from build123d import *

# Parameters (mm, degrees)
EXTRUDE_670_DEPTH        = 1730
SKETCH_2_W               = 49
SKETCH_2_H               = 55.5
EXTRUDE_1_DEPTH          = 85
SKETCH_4_W               = 49
SKETCH_4_H               = 55.5
EXTRUDE_3_DEPTH          = 95
SKETCH_9_R               = 23.5
CUT_EXTRUDE_5_DEPTH      = 3
SKETCH_10_R              = 6
EXTRUDE_4_DEPTH          = 28
CHAMFER_1_SIZE           = 1
PATTERN_CIRCULAR_1_COUNT = 4


with BuildPart() as part:
    # 草图1 → Extrude 670 (new body)
    with BuildSketch(Plane.XY):
        Polygon((15, 50), (15, 42), (35, 42), (35, 50), (50, 50), (50, 20), (42, 20), (42, 10), (50, 10), (50, 0), (0, 0), (0, 10), (8, 10), (8, 20), (0, 20), (0, 50), align=None)
    extrude(amount=EXTRUDE_670_DEPTH)

    # 草图2 → 凸台-拉伸1 (add)
    with BuildSketch(Plane.XY.offset(1730)):
        with Locations((25, 27.75)):
            Rectangle(SKETCH_2_W, SKETCH_2_H)
    extrude(amount=EXTRUDE_1_DEPTH)

    # 草图4 → 凸台-拉伸3 (add)
    with BuildSketch(Plane(origin=(0, 0, 0), x_dir=(-1, 0, 0), z_dir=(0, 0, -1))):
        with Locations((-25, 27.75)):
            Rectangle(SKETCH_4_W, SKETCH_4_H)
    extrude(amount=EXTRUDE_3_DEPTH)

    # 草图9 → 切除-拉伸5 (cut)
    with BuildSketch(Plane(origin=(49.5, 0, 0), x_dir=(0, 0, -1), z_dir=(1, 0, 0))):
        with Locations((56, 27.75)):
            Circle(SKETCH_9_R)
    extrude(amount=-CUT_EXTRUDE_5_DEPTH, mode=Mode.SUBTRACT)

    # 草图10 → 凸台-拉伸4 (add)
    with BuildSketch(Plane(origin=(46.5, 0, 0), x_dir=(0, 0, -1), z_dir=(1, 0, 0))):
        with Locations((56, 27.75)):
            Circle(SKETCH_10_R)
    extrude(amount=EXTRUDE_4_DEPTH)

    # 倒角1
    chamfer_1_edges = [part.edges().sort_by_distance(p)[0] for p in [
        (74.5, 27.75, -50),
    ]]
    chamfer(chamfer_1_edges, length=CHAMFER_1_SIZE)

    # 草图12 → M5 螺纹孔1 (revolve, cut)
    with BuildSketch(Plane(origin=(50, 47.75, -76), x_dir=(0, 0, -1), z_dir=(0, 1, 0))):
        Polygon((0, 0), (0, 15.2618073), (2.1, 14), (2.1, 10), (2.5, 10), (2.5, 0), align=None)
    hole_wizard_m5_1 = revolve(axis=Axis((56.35, 47.75, -76), (-1, 0, 0)), mode=Mode.SUBTRACT)

    # 阵列(圆周)1: M5 螺纹孔1 ×4 about axis
    pattern_circular_1_axis = Axis((0, 27.75, -56), (1, 0, 0))
    for i in range(1, PATTERN_CIRCULAR_1_COUNT):
        add(hole_wizard_m5_1.rotate(pattern_circular_1_axis, i * 360 / PATTERN_CIRCULAR_1_COUNT), mode=Mode.SUBTRACT)


solid = part.part
The listing builds one solid part. Answer for the finished solid, in the listing's coordinates (mm). Coordinates: 2 decimals unless noted, no trailing zeros. Loops run counter-clockwise (first coordinate to the right, second up) from the corner with the lowest first, then second, coordinate; pieces in that order, holes last.
1) Determine the mould class of faces 1 (the face through (25, 28, 1815)), 2 (the face through (48.02, 13.45, -37.35)), 3 (the face through (46.5, 23, -61)), 4 (the face through (49.5, 27, 1772)) for opening direction Z: pulls with the +Z half, pulls with the -Z half, needs draft (parallel to the pull), parting line crosses it, or undercut.
2) Flat-ended cylindrical pins translate along their axes: pin 1 Ø4 at (y, z) = (7, -76) entering from +X; pin 2 Ø4.5 at (y, z) = (47.75, -36) entering from -X; pin 3 Ø12 at (x, z) = (39, 1116.5) entering from +Y. Find the tip coordinate at first contact, or state that the pin passes through.
3) Find the intervals of material crossed by L1, parallel to Y at x = 42.75, z = -36; L2, parallel to Z at x = 38.5, y = 7.75; L3, parallel to Z at x = 48, y = 27, in increasing order.
4) Find section A-A on z = 497. Write down the section's boundary in (x, y).
Values:
1. face 1: pulls with the +Z half
1. face 2: undercut
1. face 3: undercut
1. face 4: needs draft
2. pin 1: stops at x = 49.5
2. pin 2: stops at x = 0.5
2. pin 3: stops at y = 50
3. L1: y = 0 to 5.25, 10.25 to 45.25, 50.25 to 55.5
3. L2: z = -95 to -78.1, -73.9 to -38.1, -33.9 to 1815
3. L3: z = -95 to -79.49, -61.95 to -50.05, -32.51 to 1815
4. outline: (0, 0) - (50, 0) - (50, 10) - (42, 10) - (42, 20) - (50, 20) - (50, 50) - (35, 50) - (35, 42) - (15, 42) - (15, 50) - (0, 50) - (0, 20) - (8, 20) - (8, 10) - (0, 10) - close
